Part print with two shaded views. Sizes in mm from the minimum x, y, z corner. A direction names the side the tool comes from. Give positions to 0.01 mm unless a question says otherwise; leave off trailing zeros. Write each loop counter-clockwise with the first axis right and the second up, starting at its lowest first coordinate (ties: lowest second). Pieces come first, ordered by that corner, then holes.
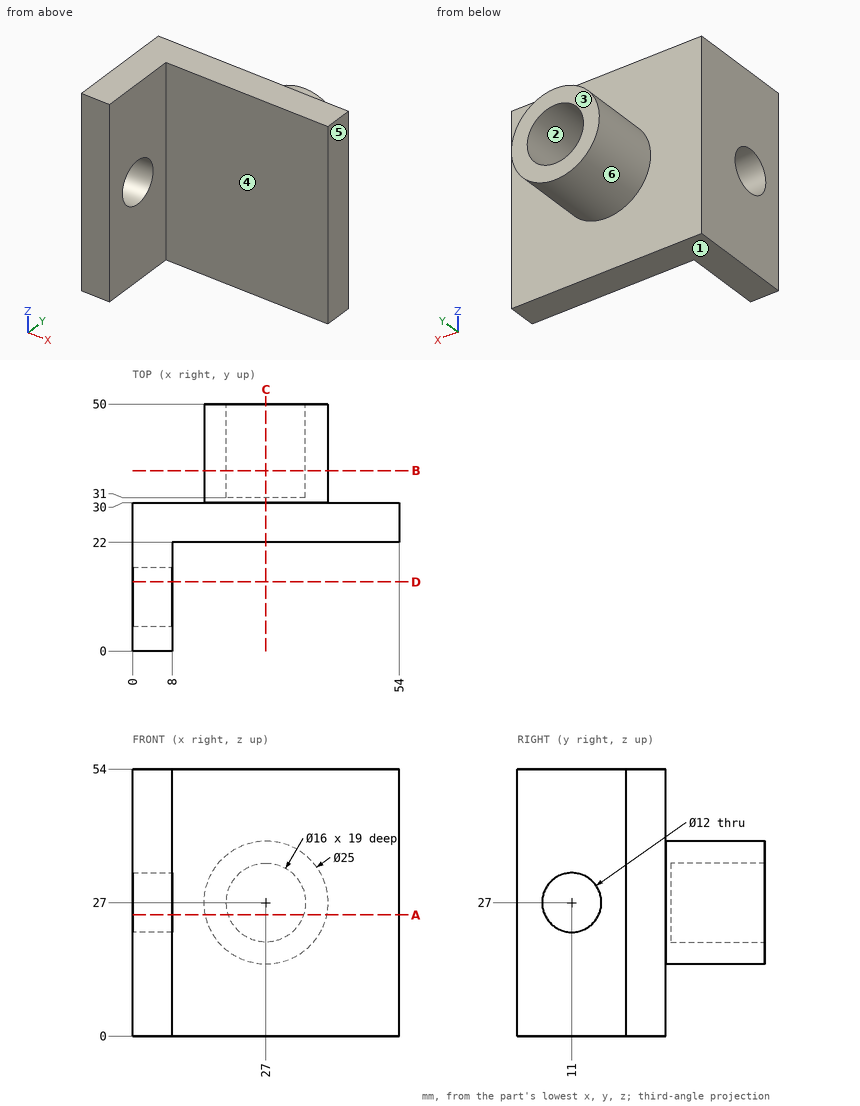
1) Saw through at C-C (x = 27). Write the cut outline in (y, z).
Check result:
outline: (22, 0) - (30, 0) - (30, 14.5) - (50, 14.5) - (50, 19) - (31, 19) - (31, 35) - (50, 35) - (50, 39.5) - (30, 39.5) - (30, 54) - (22, 54) - close
2) Saw through at A-A (z = 24.5). Write the cut outline in (x, y), and give its area (3 significant figures).
Check result:
outline: (0, 0) - (8, 0) - (8, 5.55) - (0, 5.55) - close; (0, 16.45) - (8, 16.45) - (8, 22) - (54, 22) - (54, 30) - (39.25, 30) - (39.25, 50) - (34.6, 50) - (34.6, 31) - (19.4, 31) - (19.4, 50) - (14.75, 50) - (14.75, 30) - (0, 30) - close
area: 722 mm2
3) Saw through at B-B (y = 36.5). Write the cut outline in (x, z).
Check result:
outline: circle Ø25 at (27, 27); hole circle Ø16 at (27, 27)
4) Mould opens along Z. For the marked faces 1, 2 and 3 say: +Z half, -Z half, draft (parallel to the pull), parting line (faces both ways), or undercut.
Check result:
face 1: -Z half
face 2: undercut
face 3: draft
5) Flat gauge pins, fed straight in: P1, Ø5, axis at x = 29.5, z = 28, coming from the +Y side; P2, Ø18.5, axis at x = 27, z = 27, coming from the -Y side; P3, Ø17.5, axis at y = 8, z = 39.5, coming from the +X side. Where does each tip first touch, or does it go through?
Check result:
P1: stops at y = 31
P2: stops at y = 22
P3: stops at x = 8
6) Drill centre lines: L1, parallel to Y at x = 42.5, z = 3.5; L2, parallel to X at y = 17.5, z = 15; L3, parallel to Z at x = 21.5, y = 45.5. Where is each one in solid material? Low to high.
Check result:
L1: y = 22 to 30
L2: x = 0 to 8
L3: z = 15.78 to 21.19, 32.81 to 38.22
7) Saw through at D-D (y = 14). Write the cut outline in (x, z).
Check result:
outline: (0, 0) - (8, 0) - (8, 21.8) - (0, 21.8) - close; (0, 32.2) - (8, 32.2) - (8, 54) - (0, 54) - close
8) 3-axis set-ups, long thin cutter, end or side, ignore diameter. For the marked faces 4, 5 and 6: which of +Z, -Z, +X, -X, +Y, -Y reach the whole face in a straight line?
Check result:
face 4: +Z, -Z, +X, -Y
face 5: +Z, -Z, +X, +Y, -Y
face 6: +Y
